For this review, use the dimensioned drawing (mm, ordinates from the lowest corner) and the shaded views. A direction names the side the tool comes from. Give positions to 0.01 mm unless a question says otherwise; leave off trailing zeros. Write each loop counter-clockwise with the first axis right and the second up, starting at its lowest first coordinate (ties: lowest second). Pieces come first, ordered by that corner, then holes.
1) We need section C-C on z = 2.3. Give the boundary of the cut face in (x, y), and give its area (4 significant figures).
2) We need section A-A on x = 60. Give the boundary of the cut face in (y, z).
3) Machinability: for the marked faces 1 and 2, which of the approach directions +Z, -Z, +X, -X, +Y, -Y give a long, thin tool a straight path to every point of the face, cutting with its end or side? Answer none if there is none.
4) We need section D-D on y = 29. Give the boundary of the cut face in (x, z) (1 decimal).
5) Wall thickness on line 1 along X through (y, z) = (33, 3.05) (1 decimal); line 2 along X through (y, z) = (27, 4.7) (1 decimal); line 3 along X through (y, z) = (26, 4) (1 decimal): over which ranges is each line inside the solid? List them lowest first.
6) For P1, Ø2, axis at y = 14, z = 3, coming from the -X side; P2, Ø2.5, axis at y = 38, z = 2, coming from the +X side, all flat-tipped, find the tip position at first contact; note any pin that passes through.
7) We need section B-B on y = 33. Give the boundary of the cut face in (x, z), and give its area (3 significant figures).
8) Draft analysis for pull direction X (two halves, no side actions). For the marked faces 3, 4, 5 and 6, state which applies: pulls with the +X half, pulls with the -X half, needs draft (parallel to the pull), parting line crosses it, or undercut.
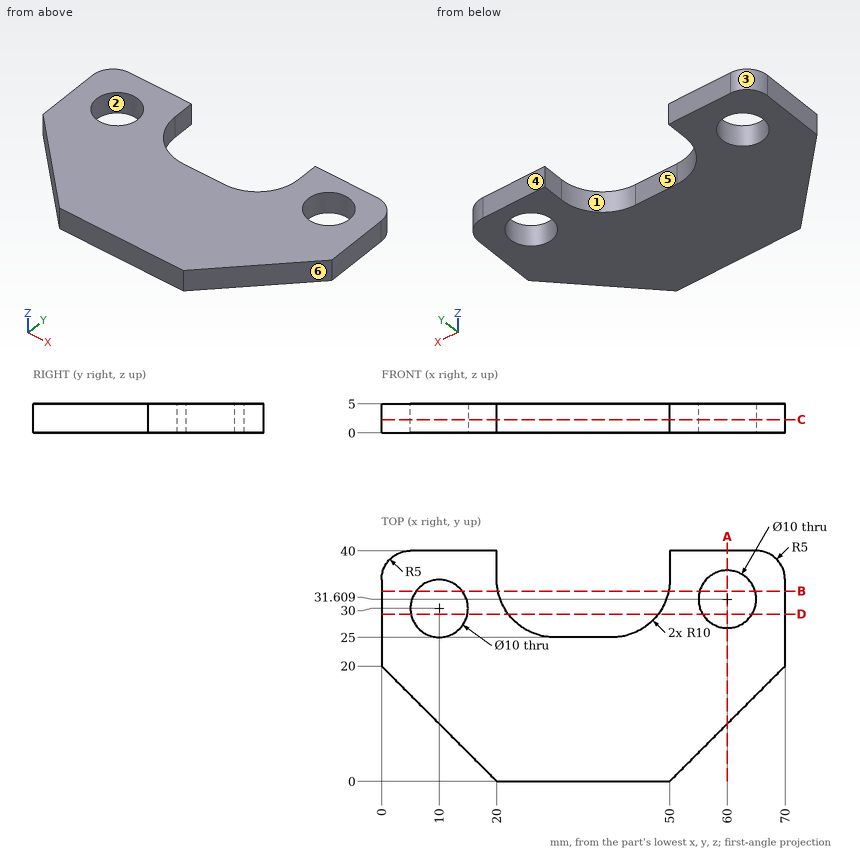
Results list:
1. outline: (0, 20) - (20, 0) - (50, 0) - (70, 20) - (70, 35) arc R5 ccw to (65, 40) - (50, 40) - (50, 35) arc R10 cw to (40, 25) - (30, 25) arc R10 cw to (20, 35) - (20, 40) - (5, 40) arc R5 ccw to (0, 35) - close; hole circle Ø10 at (10, 30); hole circle Ø10 at (60, 31.61)
1. area: 1,825 mm2
2. outline: (10, 0) - (26.61, 0) - (26.61, 5) - (10, 5) - close; (36.61, 0) - (40, 0) - (40, 5) - (36.61, 5) - close
3. face 1: +Z, -Z, +Y
3. face 2: +Z, -Z
4. outline: (0, 0) - (5.1, 0) - (5.1, 5) - (0, 5) - close; (14.9, 0) - (22, 0) - (22, 5) - (14.9, 5) - close; (48, 0) - (55.7, 0) - (55.7, 5) - (48, 5) - close; (64.3, 0) - (70, 0) - (70, 5) - (64.3, 5) - close
5. line 1: x = 0 to 6, 14 to 20.2, 49.8 to 55.2, 64.8 to 70
5. line 2: x = 0 to 6, 14 to 24, 46 to 58.1, 61.9 to 70
5. line 3: x = 0 to 7, 13 to 25.6, 44.4 to 70
6. P1: stops at x = 5
6. P2: stops at x = 69.68
7. outline: (0, 0) - (6, 0) - (6, 5) - (0, 5) - close; (14, 0) - (20.2, 0) - (20.2, 5) - (14, 5) - close; (49.8, 0) - (55.2, 0) - (55.2, 5) - (49.8, 5) - close; (64.8, 0) - (70, 0) - (70, 5) - (64.8, 5) - close
7. area: 114 mm2
8. face 3: pulls with the -X half
8. face 4: needs draft
8. face 5: undercut
8. face 6: pulls with the +X half
